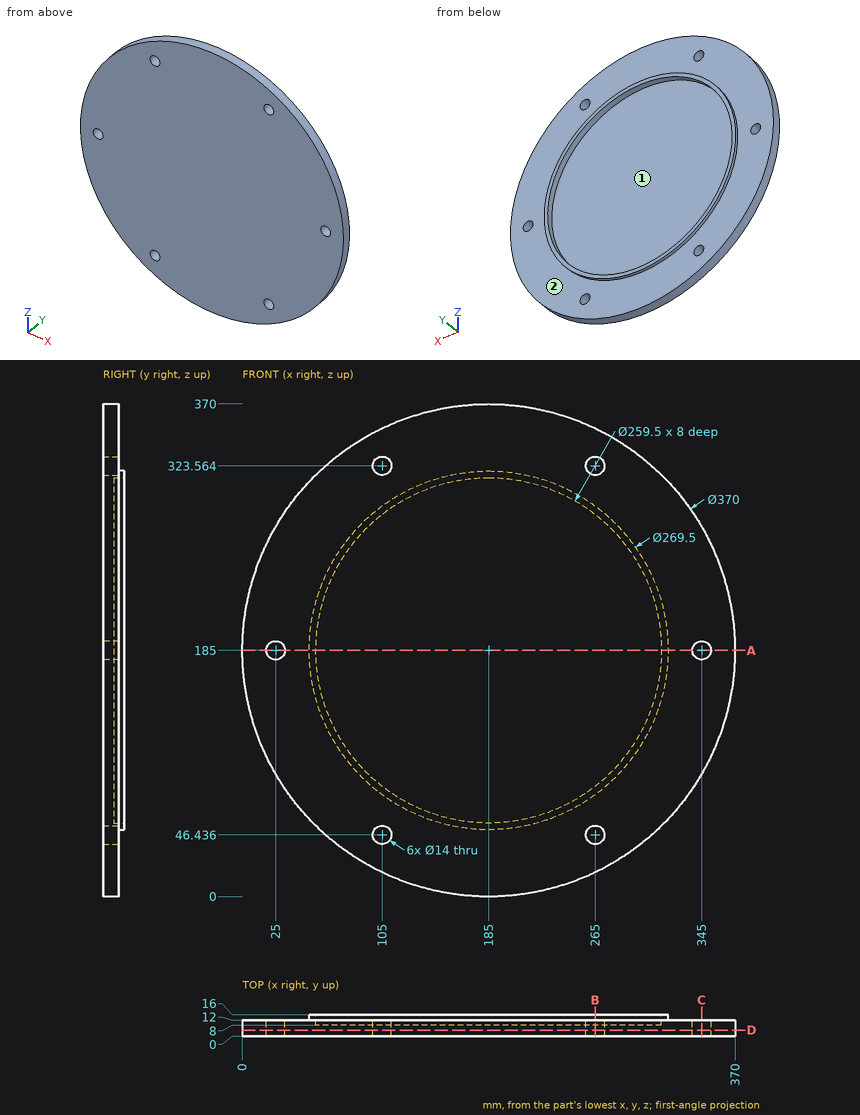
The figure shows three views and two pictorial views of one solid part (mm, origin at its lowest corner). Answer the questions. Give positions to 0.01 mm unless a question says otherwise; leave off trailing zeros. Loops run counter-clockwise (first coordinate to the right, second up) from the corner with the lowest first, then second, coordinate; pieces in that order, holes last. Notation, with made-up numbers: M -4,-4.5 L 53,-4.5 A17 cw 53,25.5 Z; hole C 13,-26.5 d8. An arc over 180 degrees is marked long. Write each question's results on one line, items separated by ' | '.
1. Section D-D on y = 4.5 is taken. Give the vertices of the cut face in (x, z).
Values:
outline: C 185,185 d370; hole C 25,185 d14; hole C 105,46.44 d14; hole C 105,323.56 d14; hole C 265,46.44 d14; hole C 265,323.56 d14; hole C 345,185 d14
2. Section C-C on x = 345 is taken. Give the vertices of the cut face in (y, z).
Values:
outline: M 0,92.13 L 12,92.13 L 12,178 L 0,178 Z; M 0,192 L 12,192 L 12,277.87 L 0,277.87 Z
3. Straight lines are drawn through the part: line 1 (X direction, y = 3.75, z = 185); line 2 (Z direction, x = 268.5, y = 10.5); line 3 (Y direction, x = 132.5, z = 346.5). For each, find the intervals that lie inside material, in ascending order. Write a range as [from, to].
Values:
line 1: x = [0, 18], [32, 338], [352, 370] | line 2: z = [19.92, 40.37], [52.5, 85.69], [284.31, 317.5], [329.63, 350.08] | line 3: y = [0, 12]
4. The mould has two halves that part along X. Classify the marked faces 1 and 2: pulls with the +X half, pulls with the -X half, needs draft (parallel to the pull), parting line crosses it, or undercut.
Values:
face 1: undercut | face 2: needs draft
5. Section B-B on x = 265 is taken. Give the vertices of the cut face in (y, z), plus the area to 3 significant figures.
Values:
outline: M 0,18.19 L 12,18.19 L 12,39.44 L 0,39.44 Z; M 0,53.44 L 12,53.44 L 12,76.57 L 16,76.57 L 16,82.85 L 8,82.85 L 8,287.15 L 16,287.15 L 16,293.43 L 12,293.43 L 12,316.56 L 0,316.56 Z; M 0,330.56 L 12,330.56 L 12,351.81 L 0,351.81 Z | area: 2,900 mm^2
6. Given pin 1 (5 mm diameter, centred on y = 11, z = 130, fed in from +X); pin 2 (1.5 mm diameter, centred on x = 250.5, y = 5, fed in from -Z); pin 3 (4 mm diameter, centred on x = 311.5, z = 127.5, fed in from +Y), each flat-ended and moving along its own axis, determine where each tip first touches the part or whether it passes through.
Values:
pin 1: stops at x = 362.39 | pin 2: stops at z = 11.7 | pin 3: stops at y = 12
7. Section A-A on z = 185 is taken. Give the vertices of the cut face in (x, y), plus the area to 3 significant figures.
Values:
outline: M 0,0 L 18,0 L 18,12 L 0,12 Z; M 32,0 L 338,0 L 338,12 L 319.75,12 L 319.75,16 L 314.75,16 L 314.75,8 L 55.25,8 L 55.25,16 L 50.25,16 L 50.25,12 L 32,12 Z; M 352,0 L 370,0 L 370,12 L 352,12 Z | area: 3,110 mm^2
